The listing builds one solid part. Answer for the finished solid, in the listing's coordinates (mm). A direction names the side the tool comes from. Coordinates: 2 decimals unless noted, no trailing zeros. Loops run counter-clockwise (first coordinate to the right, second up) from the corner with the lowest first, then second, coordinate; pieces in that order, holes last. Notation, with made-up numbers: (15.5, 41.5) - (51.5, 41.5) arc R32 ccw to (51.5, 68.5) - close; hole circle Ø8 at (-35, 55). An arc over 180 degrees is marked (long way). Put each result on its own line as item: value.
```python
from build123d import *

# Parameters (mm, degrees)
BOSS_EXTRUDE1_DEPTH = 10
CUT_EXTRUDE1_DEPTH  = 5


with BuildPart() as part:
    # Sketch2 → Boss-Extrude1 (new, symmetric)
    with BuildSketch(Plane.XY):
        with BuildLine():
            Line((-155, 32.5), (155, 32.5))
            ThreePointArc((155, 32.5), (187.376327688, 2.832561639), (160.643565774, -32.006251973))
            Line((160.643565774, -32.006251973), (125.524931981, -38.198614636))
            Line((125.524931981, -38.198614636), (-125.524931981, -38.198614636))
            Line((-125.524931981, -38.198614636), (-160.643565774, -32.006251973))
            ThreePointArc((-160.643565774, -32.006251973), (-187.376327688, 2.832561639), (-155, 32.5))
        make_face()
        with BuildLine():
            Line((-155, 20.5), (155, 20.5))
            ThreePointArc((155, 20.5), (175.421991311, 1.786692726), (158.559787642, -20.188558937))
            Line((158.559787642, -20.188558937), (124.475068019, -26.198614636))
            Line((124.475068019, -26.198614636), (-124.475068019, -26.198614636))
            Line((-124.475068019, -26.198614636), (-158.559787642, -20.188558937))
            ThreePointArc((-158.559787642, -20.188558937), (-175.421991311, 1.786692726), (-155, 20.5))
        make_face(mode=Mode.SUBTRACT)
    extrude(amount=BOSS_EXTRUDE1_DEPTH, both=True)

    # Sketch8 → Cut-Extrude1 (cut, symmetric)
    with BuildSketch(Plane.XY):
        with BuildLine():
            Line((125.437443318, -37.198614636), (160.469917597, -31.02144422))
            ThreePointArc((160.469917597, -31.02144422), (186.38013299, 2.745405897), (155, 31.5))
            Line((155, 31.5), (-155, 31.5))
            ThreePointArc((-155, 31.5), (-186.38013299, 2.745405897), (-160.469917597, -31.02144422))
            Line((-160.469917597, -31.02144422), (-125.437443318, -37.198614636))
            Line((-125.437443318, -37.198614636), (125.437443318, -37.198614636))
        make_face()
    extrude(amount=CUT_EXTRUDE1_DEPTH, both=True, mode=Mode.SUBTRACT)


solid = part.part
```
1) The part is cut by section A-A (x = -41). Give the vertices of the cut face in (y, z).
Found:
outline: (-38.2, -10) - (-26.2, -10) - (-26.2, -5) - (-37.2, -5) - (-37.2, 5) - (-26.2, 5) - (-26.2, 10) - (-38.2, 10) - close; (20.5, -10) - (32.5, -10) - (32.5, 10) - (20.5, 10) - (20.5, 5) - (31.5, 5) - (31.5, -5) - (20.5, -5) - close
2) For faces 5 (the face through (187.31, 3.5, 0.14)), 6 (the face through (-175.455, 1.362, 7.535)), 7 (the face through (-1, 25, 5)), determine the directions among +Z, -Z, +X, -X, +Y, -Y from which every point of the face is accessible in a straight line to the end or side of a thin tool.
Found:
face 5: +Z, -Z, +X
face 6: +Z, -Z
face 7: none
3) Each of these flat-tipped pins is pushed along its axis until it touches: pin 1 (8 mm diameter, centred on y = 4.5, z = 4, fed in from -X); pin 2 (6 mm diameter, centred on y = -23, z = 3.5, fed in from -X); pin 3 (5 mm diameter, centred on y = 19, z = -5, fed in from +X). Where does it stop, or does it pass through?
Found:
pin 1: stops at x = -187.5
pin 2: stops at x = -180.62
pin 3: stops at x = 183
4) The part is cut by section C-C (y = 11.5). Give the vertices of the cut face in (x, z), and give its area (3 significant figures).
Found:
outline: (-185.4, -10) - (-171.97, -10) - (-171.97, -5) - (-184.33, -5) - (-184.33, 5) - (-171.97, 5) - (-171.97, 10) - (-185.4, 10) - close; (171.97, -10) - (185.4, -10) - (185.4, 10) - (171.97, 10) - (171.97, 5) - (184.33, 5) - (184.33, -5) - (171.97, -5) - close
area: 290 mm^2
5) The part is cut by section B-B (z = -0.75). Give the vertices of the cut face in (x, y).
Found:
outline: (-160.64, -32.01) - (-125.52, -38.2) - (125.52, -38.2) - (160.64, -32.01) arc R32.5 ccw to (155, 32.5) - (-155, 32.5) arc R32.5 ccw to start; hole (-160.47, -31.02) - (-125.44, -37.2) - (125.44, -37.2) - (160.47, -31.02) arc R31.5 ccw to (155, 31.5) - (-155, 31.5) arc R31.5 ccw to start
6) For a pull along X with two mould halves and no side action, classify faces 1 (the face through (-2, -37.199, 0)), 2 (the face through (143.33, -35.06, 0.14)), 3 (the face through (-142.838, -35.146, 0.14)), 4 (the face through (1, -29, 10)) as pulls with the +X half, pulls with the -X half, needs draft (parallel to the pull), parting line crosses it, or undercut.
Found:
face 1: undercut
face 2: pulls with the +X half
face 3: pulls with the -X half
face 4: needs draft
7) Straight lines are drawn through the part: L1, parallel to Y at x = 101, z = 2; L2, parallel to Y at x = 59, z = 5.5; L3, parallel to Z at x = -49.5, y = 29. For each, find the intervals that lie inside material, in ascending order. Write a range as [from, to].
Found:
L1: y = [-38.2, -37.2], [31.5, 32.5]
L2: y = [-38.2, -26.2], [20.5, 32.5]
L3: z = [-10, -5], [5, 10]
